from build123d import *

# Parameters (mm, degrees)
BASE_BLOCK_SKETCH_W         = 108
BASE_BLOCK_SKETCH_H         = 80
BASE_BLOCK_108X80X40_DEPTH  = 40
BOX_POCKET_SKETCH_W         = 28
BOX_POCKET_SKETCH_H         = 32
THROUGH_CUT_40_DEPTH        = 40
BOX_POCKET_35_DEEP_DEPTH    = 35
FORK_LUGS_DEPTH             = 80
LUG_WEB_16_DEPTH            = 16
POCKET_START                = -16
POCKET_INFILL_BOSS_16_DEPTH = 16
PIN_BORE_SKETCH_R           = 12.5
PIN_BORE_SKETCH_R_2         = 8
PIN_BORES_16_DEPTH          = 117.086174887
TOP_HOLES_SKETCH_R          = 4
TOP_HOLES_8_DEPTH           = 38
BASE_CORNER_FILLETS_R10_R   = 10
LOWER_LUG_SKETCH_R          = 4
LOWER_LUG_BOSS_8_DEPTH      = 8


with BuildPart() as part:
    # Base Block Sketch → Base Block 108x80x40 (new body)
    with BuildSketch(Plane(origin=(0, 0, 0), x_dir=(1, 0, 0), z_dir=(0, 1, 0))):
        Rectangle(BASE_BLOCK_SKETCH_W, BASE_BLOCK_SKETCH_H)
    extrude(amount=BASE_BLOCK_108X80X40_DEPTH)

    # Box Pocket Sketch → Through Cut 40 (cut)
    with BuildSketch(Plane(origin=(0, 40, 0), x_dir=(1, 0, 0), z_dir=(0, 1, 0))):
        with Locations((40, -16)):
            Rectangle(BOX_POCKET_SKETCH_W, BOX_POCKET_SKETCH_H)
        with Locations((40, 16)):
            Rectangle(BOX_POCKET_SKETCH_W, BOX_POCKET_SKETCH_H)
    extrude(amount=-THROUGH_CUT_40_DEPTH, mode=Mode.SUBTRACT)

    # Sketch3_3 → Box Pocket 35 Deep (cut)
    with BuildSketch(Plane(origin=(0, 40, 0), x_dir=(1, 0, 0), z_dir=(0, 1, 0))):
        with BuildLine():
            Line((-22, -32), (26, -32))
            Line((26, -32), (26, 32))
            Line((26, 32), (-22, 32))
            ThreePointArc((-22, 32), (-27.656854249, 29.656854249), (-30, 24))
            ThreePointArc((-30, 24), (-32.343145751, 18.343145751), (-38, 16))
            ThreePointArc((-38, 16), (-43.656854249, 13.656854249), (-46, 8))
            Line((-46, 8), (-46, -8))
            ThreePointArc((-46, -8), (-43.656854249, -13.656854249), (-38, -16))
            ThreePointArc((-38, -16), (-32.343145751, -18.343145751), (-30, -24))
            ThreePointArc((-30, -24), (-27.656854249, -29.656854249), (-22, -32))
        make_face()
    extrude(amount=-BOX_POCKET_35_DEEP_DEPTH, mode=Mode.SUBTRACT)

    # Fork Lug Sketch → Fork Lugs (add)
    with BuildSketch(Plane.XY.offset(40)):
        with BuildLine():
            Line((-12.627416998, 0), (32.627416998, 0))
            ThreePointArc((32.627416998, 0), (26.095444351, -3.381197846), (25.084944665, -10.666666667))
            ThreePointArc((25.084944665, -10.666666667), (10, -32), (-5.084944665, -10.666666667))
            ThreePointArc((-5.084944665, -10.666666667), (-6.095444351, -3.381197846), (-12.627416998, 0))
        make_face()
    extrude(amount=-FORK_LUGS_DEPTH)

    # Lug Web Sketch → Lug Web 16 (add)
    with BuildSketch(Plane.XY.offset(40)):
        with BuildLine():
            Line((37.663470885, 31.537669456), (15.39, 0))
            Line((15.39, 0), (26, 0))
            Line((26, 0), (26.095444351, -3.381197846))
            ThreePointArc((26.095444351, -3.381197846), (28.949810251, -0.895409328), (32.627416998, 0))
            Line((32.627416998, 0), (54, 0))
            ThreePointArc((54, 0), (71.758848346, 29.199092642), (37.663470885, 31.537669456))
        make_face()
    extrude(amount=-LUG_WEB_16_DEPTH)

    # Pocket Infill Sketch → Pocket Infill Boss 16 (add)
    with BuildSketch(Plane(origin=(0, 0, -40), x_dir=(-1, 0, 0), z_dir=(0, 0, -1)).offset(POCKET_START)):
        with BuildLine():
            Line((-32.627416998, 0), (-54, 0))
            ThreePointArc((-54, 0), (-74, 20), (-54, 40))
            ThreePointArc((-54, 40), (-44.800907358, 37.758848346), (-37.663470885, 31.537669456))
            Line((-37.663470885, 31.537669456), (-18.921248705, 5))
            Line((-18.921248705, 5), (-26, 5))
            Line((-26, 5), (-26, -3.519225074))
            ThreePointArc((-26, -3.519225074), (-28.87549745, -0.934371953), (-32.627416998, 0))
        make_face()
    extrude(amount=POCKET_INFILL_BOSS_16_DEPTH)

    # Pin Bore Sketch → Pin Bores _16 (cut, through all)
    with BuildSketch(Plane.XY.offset(40)):
        with Locations((54, 20)):
            Circle(PIN_BORE_SKETCH_R)
        with Locations((10, -16)):
            Circle(PIN_BORE_SKETCH_R_2)
    extrude(amount=-PIN_BORES_16_DEPTH, mode=Mode.SUBTRACT)

    # Top Holes Sketch → Top Holes _8 (cut)
    with BuildSketch(Plane(origin=(0, 40, 0), x_dir=(1, 0, 0), z_dir=(0, 1, 0))):
        with Locations(Location((-38, 24, 0), (0, 0, 270))):
            Circle(TOP_HOLES_SKETCH_R)
        with Locations(Location((-38, -24, 0), (0, 0, 270))):
            Circle(TOP_HOLES_SKETCH_R)
    extrude(amount=-TOP_HOLES_8_DEPTH, mode=Mode.SUBTRACT)

    # Base Corner Fillets R10
    base_corner_fillets_r10_edges = [part.edges().sort_by_distance(p)[0] for p in [
        (-54, 20, 40),
        (-54, 20, -40),
    ]]
    fillet(base_corner_fillets_r10_edges, radius=BASE_CORNER_FILLETS_R10_R)

    # Lower Lug Sketch → Lower Lug Boss 8 (add)
    with BuildSketch(Plane.ZY.offset(54)):
        with BuildLine():
            Line((-8, 16), (-8, 0))
            Line((-8, 0), (8, 0))
            Line((8, 0), (8, 16))
            ThreePointArc((8, 16), (0, 24), (-8, 16))
        make_face()
        with Locations((0, 16)):
            Circle(LOWER_LUG_SKETCH_R, mode=Mode.SUBTRACT)
    extrude(amount=LOWER_LUG_BOSS_8_DEPTH)


solid = part.part
The model under review builds one solid part; all positions refer to its coordinate system, in mm. A direction names the side the tool comes from. Coordinates: 2 decimals unless noted, no trailing zeros. Loops run counter-clockwise (first coordinate to the right, second up) from the corner with the lowest first, then second, coordinate; pieces in that order, holes last. Notation, with made-up numbers: (-10, -12) -> (37, -12) arc R18 cw to (37, -7) -> close; hole circle Ø8 at (32.5, 80). An arc over 180 degrees is marked (long way). Use a Markdown table: item, result. Add a question column.
1. Machinability: for faces 1 (the face through (-54, 16, 0)), 2 (the face through (43, 0, -32)), 3 (the face through (7, 23, 32)), which of the approach directions +Z, -Z, +X, -X, +Y, -Y give a long, thin tool a straight path to every point of the face, cutting with its end or side? Answer none if there is none.
2. Add section A-A on y = -16. Write out the cut boundary in (x, z), plus the area to 3 significant figures.
3. Add section D-D on y = 22.5. Give the number of separate pieces and of enclosed holes in the cut face, plus the area to 3 significant figures.
4. To check wall thickness, follow line 1 (Y direction, x = 54, z = -34); line 2 (Z direction, x = 60.5, y = 7); line 3 (Y direction, x = -59, z = 0). State the ranges of each line that lie inside material, in increasing order.
5. Clearance check with flat-ended pins moving along their axes: pin 1 Ø12 at (y, z) = (-2, -23) entering from -X; pin 2 Ø7.5 at (x, z) = (29.5, -8.5) entering from +Y; pin 3 Ø17.5 at (x, z) = (38, 33) entering from -Y. State where each tip first meets the part, or that it passes through.
6. Add section C-C on z = 10. Write out the cut boundary in (x, y), plus the area to 3 significant figures.
7. Draft analysis for pull direction Y (two halves, no side actions). For faces 4 (the face through (3.651, -20.868, 0.56)), 5 (the face through (-32, 0, -1)), 6 (the face through (40, 16, 24)), state which applies: pulls with the +Y half, pulls with the -Y half, needs draft (parallel to the pull), parting line crosses it, or undercut.
8. Add section B-B on x = -20.5. Write out the cut boundary in (y, z).
Returned:
| question | item | result |
|---|---|---|
| 1 | face 1 | -X |
| 1 | face 2 | +Z, -Z, +X, -Y |
| 1 | face 3 | +Y |
| 2 | outline | (-6, -40) -> (2, -40) -> (2, 40) -> (-6, 40) -> close; (18, -40) -> (26, -40) -> (26, 40) -> (18, 40) -> close |
| 2 | area | 1,280 mm² |
| 3 | separate pieces | 3 |
| 3 | enclosed holes | 2 |
| 3 | area | 2,930 mm² |
| 4 | line 1 | y = 0 to 7.5, 32.5 to 40 |
| 4 | line 2 | z = -40 to -24, 24 to 40 |
| 4 | line 3 | y = 0 to 12, 20 to 24 |
| 5 | pin 1 | stops at x = -54 |
| 5 | pin 2 | stops at y = 5 |
| 5 | pin 3 | stops at y = -0.75 |
| 6 | outline | (-54, 0) -> (-12.63, 0) arc R8 cw to (-5.08, -10.67) arc R16 ccw (long way) to (25.08, -10.67) arc R8 cw to (32.63, 0) -> (26, 0) -> (26, 5) -> (-45.75, 5) -> (-45.75, 40) -> (-54, 40) -> close; hole circle Ø16 at (10, -16) |
| 6 | area | 1,400 mm² |
| 7 | face 4 | undercut |
| 7 | face 5 | pulls with the -Y half |
| 7 | face 6 | needs draft |
| 8 | outline | (0, -40) -> (40, -40) -> (40, -32) -> (5, -32) -> (5, 32) -> (40, 32) -> (40, 40) -> (0, 40) -> close |
